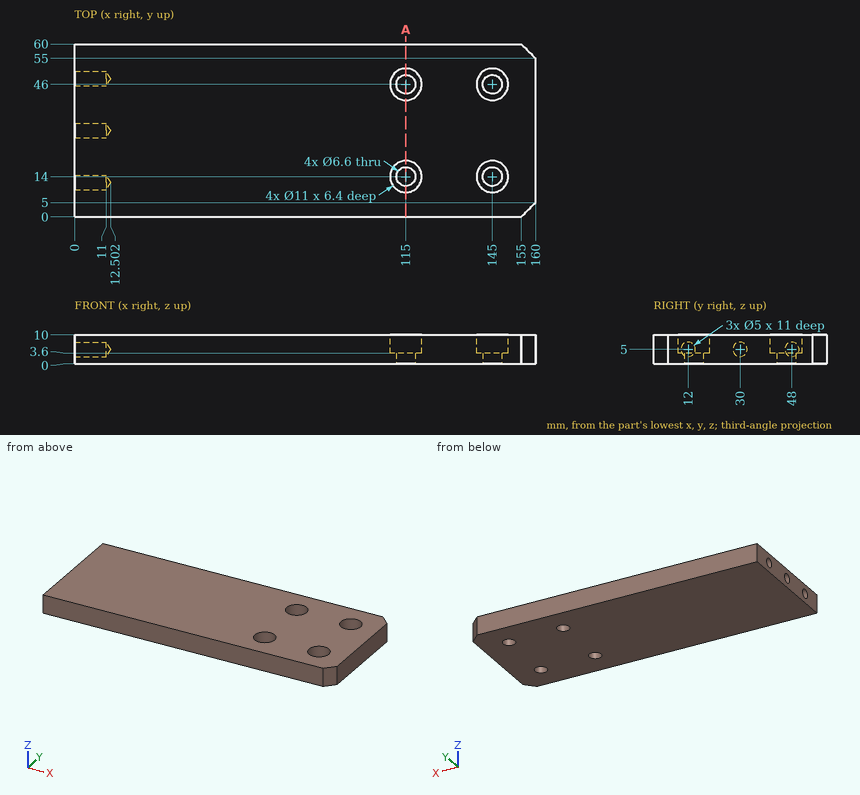
Study the drawing (mm; zero at the part's minimum x, y, z) and answer. Coordinates: 2 decimals unless noted, no trailing zeros. Write each loop counter-clockwise with the first axis right and the second up, starting at its lowest first coordinate (ties: lowest second). Pieces come first, ordered by that corner, then holes.
Q1. Find the intervals of material crossed by line 1 (Y direction, x = 145, z = 8.5); line 2 (Y direction, x = 145, z = 2.35); line 3 (X direction, y = 51, z = 9), in increasing order.
Q2. A cutting plane is placed at A-A, the plane x = 115. Give the vertices of the cut face in (y, z), then the cut area to 3 significant figures.
Q3. Each of these flat-tipped pins is pushed along its axis until it touches: pin 1 Ø3.5 at (x, y) = (117.5, 45.5) entering from +Z; pin 2 Ø4 at (y, z) = (48, 5) entering from -X. Where does it stop, or does it pass through?
Findings below:
1. line 1: y = 0 to 8.5, 19.5 to 40.5, 51.5 to 60
1. line 2: y = 0 to 10.7, 17.3 to 42.7, 49.3 to 60
1. line 3: x = 0 to 112.71, 117.29 to 142.71, 147.29 to 160
2. outline: (0, 0) - (10.7, 0) - (10.7, 3.6) - (8.5, 3.6) - (8.5, 10) - (0, 10) - close; (17.3, 0) - (42.7, 0) - (42.7, 3.6) - (40.5, 3.6) - (40.5, 10) - (19.5, 10) - (19.5, 3.6) - (17.3, 3.6) - close; (49.3, 0) - (60, 0) - (60, 10) - (51.5, 10) - (51.5, 3.6) - (49.3, 3.6) - close
2. area: 412 mm2
3. pin 1: stops at z = 3.6
3. pin 2: stops at x = 11.3
